from build123d import *

# Parameters (mm, degrees)
BASE_PLATE_305X178X28_DEPTH    = 14
FACE_RECESS_3MM_DEPTH          = 3
END_SLOTS_PROFILE_R            = 6.963047248
END_SLOTS_PROFILE_R_2          = 6.498844098
END_SLOTS_PROFILE_R_3          = 5.742027746
END_SLOTS_PROFILE_R_4          = 6.051697443
END_U_SLOTS_CUT_DEPTH          = 38
TWO_HOLE_POCKET_CUT_DEPTH      = 179.777095848
TWO_HOLE_POCKET_CUT_DEPTH_BACK = 179.777095848


with BuildPart() as part:
    # Base Plate Profile → Base Plate 305x178x28 (new, symmetric)
    with BuildSketch(Plane.XY):
        with BuildLine():
            Line((-140, 89), (140, 89))
            ThreePointArc((140, 89), (148.838834765, 85.338834765), (152.5, 76.5))
            Line((152.5, 76.5), (152.5, -76.5))
            ThreePointArc((152.5, -76.5), (148.838834765, -85.338834765), (140, -89))
            Line((140, -89), (-140, -89))
            ThreePointArc((-140, -89), (-148.838834765, -85.338834765), (-152.5, -76.5))
            Line((-152.5, -76.5), (-152.5, 76.5))
            ThreePointArc((-152.5, 76.5), (-148.838834765, 85.338834765), (-140, 89))
        make_face()
    extrude(amount=BASE_PLATE_305X178X28_DEPTH, both=True)

    # Face Recess Profile → Face Recess 3mm (cut)
    with BuildSketch(Plane.XY.offset(14)):
        with BuildLine():
            ThreePointArc((-152.5, -76.5), (-148.838834765, -85.338834765), (-140, -89))
            Line((-140, -89), (140, -89))
            ThreePointArc((140, -89), (148.838834765, -85.338834765), (152.5, -76.5))
            Line((152.5, -76.5), (152.5, -60))
            Line((152.5, -60), (132.5, -60))
            ThreePointArc((132.5, -60), (118.5, -46), (132.5, -32))
            Line((132.5, -32), (152.5, -32))
            Line((152.5, -32), (152.5, 32))
            Line((152.5, 32), (132.5, 32))
            ThreePointArc((132.5, 32), (118.5, 46), (132.5, 60))
            Line((132.5, 60), (152.5, 60))
            Line((152.5, 60), (152.5, 76.5))
            ThreePointArc((152.5, 76.5), (148.838834765, 85.338834765), (140, 89))
            Line((140, 89), (-140, 89))
            ThreePointArc((-140, 89), (-148.838834765, 85.338834765), (-152.5, 76.5))
            Line((-152.5, 76.5), (-152.5, 60))
            Line((-152.5, 60), (-132.5, 60))
            ThreePointArc((-132.5, 60), (-118.5, 46), (-132.5, 32))
            Line((-132.5, 32), (-152.5, 32))
            Line((-152.5, 32), (-152.5, -32))
            Line((-152.5, -32), (-132.5, -32))
            ThreePointArc((-132.5, -32), (-118.5, -46), (-132.5, -60))
            Line((-132.5, -60), (-152.5, -60))
            Line((-152.5, -60), (-152.5, -76.5))
        make_face()
        with BuildLine():
            ThreePointArc((-117.5, 65), (-116.035533906, 68.535533906), (-112.5, 70))
            Line((-112.5, 70), (17.5, 70))
            ThreePointArc((17.5, 70), (21.035533906, 68.535533906), (22.5, 65))
            Line((22.5, 65), (22.5, -65))
            ThreePointArc((22.5, -65), (21.035533906, -68.535533906), (17.5, -70))
            Line((17.5, -70), (-112.5, -70))
            ThreePointArc((-112.5, -70), (-116.035533906, -68.535533906), (-117.5, -65))
            Line((-117.5, -65), (-117.5, 65))
        make_face(mode=Mode.SUBTRACT)
        Polygon((47.5, -25), (47.5, 25), (72.5, 25), (72.5, -25), (60, -25), align=None, mode=Mode.SUBTRACT)
    extrude(amount=-FACE_RECESS_3MM_DEPTH, mode=Mode.SUBTRACT)

    # End Slots Profile → End U-Slots Cut (cut)
    with BuildSketch(Plane.XY.offset(14)):
        with BuildLine():
            Line((-132.297897709, 53.151260658), (-152.5, 53.151260658))
            Line((-152.5, 53.151260658), (-152.5, 39.225166163))
            Line((-152.5, 39.225166163), (-132.297897709, 39.225166163))
            ThreePointArc((-132.297897709, 39.225166163), (-125.334850461, 46.188213411), (-132.297897709, 53.151260658))
        make_face()
        with Locations((-97.5, 55)):
            Circle(END_SLOTS_PROFILE_R)
        with Locations((2.5, 55)):
            Circle(END_SLOTS_PROFILE_R_2)
        with Locations((2.5, -55)):
            Circle(END_SLOTS_PROFILE_R_2)
        with Locations((59.398868635, 13.95239873)):
            Circle(END_SLOTS_PROFILE_R_3)
        with Locations((-97.5, -55)):
            Circle(END_SLOTS_PROFILE_R)
        with Locations((59.398868635, -13.43949496)):
            Circle(END_SLOTS_PROFILE_R_4)
    extrude(amount=-END_U_SLOTS_CUT_DEPTH, mode=Mode.SUBTRACT)

    # Hole Pocket Profile → Two-Hole Pocket Cut (cut, two sides: drawn at the far end of the back side and taken through both)
    with BuildSketch(Plane.XY.offset(14).offset(-TWO_HOLE_POCKET_CUT_DEPTH_BACK)):
        with BuildLine():
            Line((-152.5, -39), (-132.5, -39))
            ThreePointArc((-132.5, -39), (-125.5, -46), (-132.5, -53))
            Line((-132.5, -53), (-152.5, -53))
            Line((-152.5, -53), (-152.5, -39))
        make_face()
        with BuildLine():
            Line((152.5, -39), (152.5, -53))
            Line((152.5, -53), (132.5, -53))
            ThreePointArc((132.5, -53), (125.5, -46), (132.5, -39))
            Line((132.5, -39), (152.5, -39))
        make_face()
        with BuildLine():
            Line((152.5, 39), (132.5, 39))
            ThreePointArc((132.5, 39), (125.5, 46), (132.5, 53))
            Line((132.5, 53), (152.5, 53))
            Line((152.5, 53), (152.5, 39))
        make_face()
    extrude(amount=TWO_HOLE_POCKET_CUT_DEPTH + TWO_HOLE_POCKET_CUT_DEPTH_BACK, mode=Mode.SUBTRACT)


solid = part.part
Work out the finished part from the listing and answer in its coordinate system (mm). A direction names the side the tool comes from. Coordinates: 2 decimals unless noted, no trailing zeros. Write each loop counter-clockwise with the first axis right and the second up, starting at its lowest first coordinate (ties: lowest second). Pieces come first, ordered by that corner, then holes.
1. The part is cut by section C-C, the plane z = -8.75. State how many separate pieces and enclosed holes the cut face has, and give its area (3 significant figures).
Results list:
separate pieces: 1
enclosed holes: 6
area: 51,900 mm2
2. For faces 1 (the cylindrical face through (-118.503, 46.308, 12.521)), 2 (the flat face through (143, 39, 0)), 3 (the flat face through (-143, 39.225, 0)), determine the directions among +Z, -Z, +X, -X, +Y, -Y from which every point of the face is accessible in a straight line to the end or side of a thin tool.
Results list:
face 1: +Z
face 2: +Z, -Z, +X
face 3: +Z, -Z, -X
3. The part is cut by section B-B, the plane x = 2.5. Write down the section's boundary in (y, z).
Results list:
outline: (-89, -14) - (-61.5, -14) - (-61.5, 14) - (-70, 14) - (-70, 11) - (-89, 11) - close; (-48.5, -14) - (48.5, -14) - (48.5, 14) - (-48.5, 14) - close; (61.5, -14) - (89, -14) - (89, 11) - (70, 11) - (70, 14) - (61.5, 14) - close
4. The part is cut by section D-D, the plane y = -36. Write down the section's boundary in (x, z).
Results list:
outline: (-152.5, -14) - (152.5, -14) - (152.5, 14) - (122.7, 14) - (122.7, 11) - (22.5, 11) - (22.5, 14) - (-117.5, 14) - (-117.5, 11) - (-122.7, 11) - (-122.7, 14) - (-152.5, 14) - close
5. Flat-ended cylindrical pins translate along their axes: pin 1 (1.5 mm diameter, centred on x = -143.5, z = 12.5, fed in from -Y); pin 2 (0.9 mm diameter, centred on x = -58, z = 13, fed in from -Y); pin 3 (11 mm diameter, centred on x = -97.5, y = 55, fed in from -Z); pin 4 (1.5 mm diameter, centred on x = 55, z = 12, fed in from +Y). Find the tip coordinate at first contact, or state that the pin passes through.
Results list:
pin 1: stops at y = -60
pin 2: stops at y = -70
pin 3: passes through
pin 4: stops at y = 25
6. The part is cut by section A-A, the plane x = -97.5. Write down the section's boundary in (y, z), and give its area (3 significant figures).
Results list:
outline: (-89, -14) - (-61.96, -14) - (-61.96, 14) - (-70, 14) - (-70, 11) - (-89, 11) - close; (-48.04, -14) - (48.04, -14) - (48.04, 14) - (-48.04, 14) - close; (61.96, -14) - (89, -14) - (89, 11) - (70, 11) - (70, 14) - (61.96, 14) - close
area: 4,090 mm2
7. For a pull along X with two mould halves and no side action, classify faces 4 (the cylindrical face through (64.7, 11.75, 0.2)), 5 (the flat face through (-47, 1, 14)), 6 (the cylindrical face through (-125.337, 46.035, 0.196)) as +X half, -X half, draft (parallel to the pull), parting line (faces both ways), or undercut.
Results list:
face 4: undercut
face 5: draft
face 6: -X half
8. Consider line 1 along Y through (x, z) = (-97.5, -0.5); line 2 along Y through (x, z) = (60, 8.5); line 3 along X through (y, z) = (-51.5, 1). Determine where each line is inside the solid, lowest interval first.
Results list:
line 1: y = -89 to -61.96, -48.04 to 48.04, 61.96 to 89
line 2: y = -89 to -19.46, -7.42 to 8.24, 19.66 to 89
line 3: x = -128.17 to -103.52, -91.48 to -2.98, 7.98 to 128.17
